```python
from build123d import *

# Parameters (mm, degrees)
SKETCH1_W           = 60
SKETCH1_H           = 60
BOSS_EXTRUDE1_DEPTH = 60
SKETCH2_R           = 21.984754573
BOSS_EXTRUDE2_DEPTH = 60


with BuildPart() as part:
    # Sketch1 → Boss-Extrude1 (new body)
    with BuildSketch(Plane(origin=(0, 0, 0), x_dir=(1, 0, 0), z_dir=(0, 1, 0))):
        Rectangle(SKETCH1_W, SKETCH1_H)
    extrude(amount=BOSS_EXTRUDE1_DEPTH)

    # Sketch2 → Boss-Extrude2 (add)
    with BuildSketch(Plane.XY.offset(30)):
        with Locations((0, 30)):
            Circle(SKETCH2_R)
    extrude(amount=BOSS_EXTRUDE2_DEPTH)


solid = part.part
```
Read the model definition and answer for the solid it produces. Units are mm, in the model's axes. A direction names the side the tool comes from. Give positions to 0.01 mm unless a question says otherwise; leave off trailing zeros. Write each loop counter-clockwise with the first axis right and the second up, starting at its lowest first coordinate (ties: lowest second). Pieces come first, ordered by that corner, then holes. Notation, with made-up numbers: (83.5, 3.25) - (102.5, 3.25) arc R18 cw to (102.5, 18.25) - close; hole circle Ø2 at (-27.5, -27.5). An arc over 180 degrees is marked (long way). Write item = value, one per line. Start each with the question number.
Item 1: Find section C-C (z = 79). Give the vertices of the cut face in (x, y), then the cut area to 3 significant figures.
Item 2: Each of these flat-tipped pins is pushed along its axis until it touches: P1, Ø8, axis at x = 20.5, z = 38.5, coming from the +Y side; P2, Ø5, axis at y = 32.5, z = 46.5, coming from the +X side; P3, Ø12, axis at x = 19.5, z = 67, coming from the +Y side. Where does it stop, or does it pass through?
Item 3: A tool of negligible diameter and unlimited length cuts with its end or side. For faces 1 (the flat face through (-14, 50, 30)), 2 (the flat face through (-30, 30, 0)), from which of +Z, -Z, +X, -X, +Y, -Y can it reach the whole face along a straight path? Write none if from no direction.
Item 4: Find the intervals of material crossed by probe 1 along Y at (x, z) = (-0.5, 59); probe 2 along Z at (x, y) = (4, 4); probe 3 along X at (y, z) = (32.5, 58), in increasing order. Write a range as [from, to].
Item 5: Find section A-A (x = 0). Give the vertices of the cut face in (y, z), then the cut area to 3 significant figures.
Item 6: Find section B-B (y = 30). Give the vertices of the cut face in (x, z), then the cut area to 3 significant figures.
Item 7: Find section D-D (y = 55.5). Give the vertices of the cut face in (x, z), then the cut area to 3 significant figures.
Response:
q1.outline = circle Ø43.97 at (0, 30)
q1.area = 1,520 mm²
q2.P1 = 44.53
q2.P2 = 21.98
q2.P3 = 47.35
q3.face_1 = +Z
q3.face_2 = +Z, -Z, -X, +Y, -Y
q4.probe_1 = [8.02, 51.98]
q4.probe_2 = [-30, 30]
q4.probe_3 = [-21.84, 21.84]
q5.outline = (0, -30) - (60, -30) - (60, 30) - (51.98, 30) - (51.98, 90) - (8.02, 90) - (8.02, 30) - (0, 30) - close
q5.area = 6,240 mm²
q6.outline = (-30, -30) - (30, -30) - (30, 30) - (21.98, 30) - (21.98, 90) - (-21.98, 90) - (-21.98, 30) - (-30, 30) - close
q6.area = 6,240 mm²
q7.outline = (-30, -30) - (30, -30) - (30, 30) - (-30, 30) - close
q7.area = 3,600 mm²
